Part model, mm, in its own coordinate system. Coordinates: 2 decimals unless noted, no trailing zeros. Loops run counter-clockwise (first coordinate to the right, second up) from the corner with the lowest first, then second, coordinate; pieces in that order, holes last. Notation, with made-up numbers: (56.5, 12.25) -> (108.5, 12.25) arc R26 ccw to (108.5, 36.25) -> close; hole circle Ø5 at (28, -31). An arc over 180 degrees is marked (long way). Use one line per item in the form item = value. Start each with the question number.
(1) Band-saw the part on B-B on y = -0.5. Give the cut face in (x, z), then the cut area to 3 significant figures.
(2) Band-saw the part on D-D on z = 8.5. Give the cut face in (x, y).
(3) Mould opens along Z. For faces 1 (the cylindrical face through (-0.31, 0.54, 36.95)), 2 (the flat face through (2.222, -3, 29)), 3 (the flat face through (0, -1, 58)) say: +Z half, -Z half, draft (parallel to the pull), parting line (faces both ways), or undercut.
(4) Pin check, flat tips, straight feed: P1, Ø1.5, axis at x = 0, z = 27, coming from the -Y side; P2, Ø4, axis at y = 0.5, z = 40.5, coming from the -X side; P3, Ø3, axis at x = -1, z = 42.5, coming from the -Y side. Stop position of each tip, or through.
(5) Band-saw the part on C-C on x = -1.7. Give the cut face in (y, z).
(6) Band-saw the part on A-A on z = 39. Give the cut face in (x, y).
(7) Drill centre lines: L1, parallel to Z at x = -0.75, y = 2; L2, parallel to Z at x = -0.8, y = -0.25; L3, parallel to Y at x = -2.05, z = 13.5. Where is each one in solid material? Low to high. Write a range as [from, to].
```python
from build123d import *

# Parameters (mm, degrees)
EXTRUDE_1_DEPTH     = 58
SKETCH_2_R          = 2.1
CUT_EXTRUDE_1_DEPTH = 60.630319876


with BuildPart() as part:
    # 草图1 → 凸台-拉伸1 (new body)
    with BuildSketch(Plane.XY):
        with BuildLine():
            Line((-2.777777778, 6.085858586), (2.222222222, 6.085858586))
            Line((2.222222222, 6.085858586), (2.222222222, -12.914141414))
            ThreePointArc((2.222222222, -12.914141414), (0.22943144, -10.106820848), (-2.777777778, -8.430826641))
            Line((-2.777777778, -8.430826641), (-2.777777778, 6.085858586))
        make_face()
    extrude(amount=EXTRUDE_1_DEPTH)

    # 草图2 → 切除-拉伸1 (cut, through all)
    with BuildSketch(Plane.ZY.offset(2.777777778)):
        with Locations(Location((19, 0.085858586, 0), (0, 0, 270))):
            Circle(SKETCH_2_R)
        with Locations(Location((39, 0.085858586, 0), (0, 0, 270))):
            Circle(SKETCH_2_R)
    extrude(amount=-CUT_EXTRUDE_1_DEPTH, mode=Mode.SUBTRACT)


solid = part.part
```
A:
q1.outline = (-2.78, 0) -> (2.22, 0) -> (2.22, 16.98) -> (-2.78, 16.98) -> close; (-2.78, 21.02) -> (2.22, 21.02) -> (2.22, 36.98) -> (-2.78, 36.98) -> close; (-2.78, 41.02) -> (2.22, 41.02) -> (2.22, 58) -> (-2.78, 58) -> close
q1.area = 250 mm²
q2.outline = (-2.78, -8.43) arc R7.8 cw to (2.22, -12.91) -> (2.22, 6.09) -> (-2.78, 6.09) -> close
q3.face_1 = undercut
q3.face_2 = draft
q3.face_3 = +Z half
q4.P1 = -10.62
q4.P2 = -2.78
q4.P3 = -10.36
q5.outline = (-8.84, 0) -> (6.09, 0) -> (6.09, 58) -> (-8.84, 58) -> close; hole circle Ø4.2 at (0.09, 19); hole circle Ø4.2 at (0.09, 39)
q6.outline = (-2.78, -8.43) arc R7.8 cw to (2.22, -12.91) -> (2.22, -2.01) -> (-2.78, -2.01) -> close; (-2.78, 2.19) -> (2.22, 2.19) -> (2.22, 6.09) -> (-2.78, 6.09) -> close
q7.L1 = [0, 18.14], [19.86, 38.14], [39.86, 58]
q7.L2 = [0, 16.93], [21.07, 36.93], [41.07, 58]
q7.L3 = [-8.68, 6.09]
